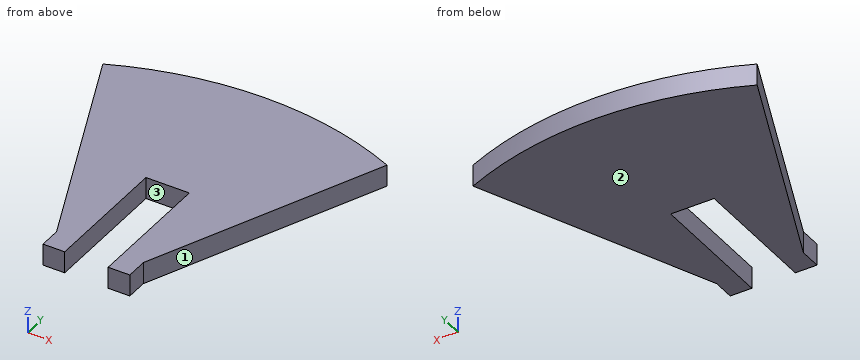
from build123d import *

# Parameters (mm, degrees)
BOSS_EXTRUDE1_DEPTH = 5
SKETCH2_W           = 20
SKETCH2_H           = 120
CUT_EXTRUDE1_DEPTH  = 10


with BuildPart() as part:
    # Sketch1 → Boss-Extrude1 (new, symmetric)
    with BuildSketch(Plane.XY):
        with BuildLine():
            Line((-65.458114903, 147.092607541), (-20, 40))
            Line((-20, 40), (-20, 30))
            Line((-20, 30), (20, 30))
            Line((20, 30), (20, 40))
            Line((20, 40), (65.458114903, 147.092607541))
            ThreePointArc((65.458114903, 147.092607541), (0, 161), (-65.458114903, 147.092607541))
        make_face()
    extrude(amount=BOSS_EXTRUDE1_DEPTH, both=True)

    # Sketch2 → Cut-Extrude1 (cut)
    with BuildSketch(Plane.XY.offset(5)):
        with Locations((0, 30)):
            Rectangle(SKETCH2_W, SKETCH2_H)
    extrude(amount=-CUT_EXTRUDE1_DEPTH, mode=Mode.SUBTRACT)


solid = part.part
Can you work these out from the model? Positions are in its coordinate system, mm. Face numbers are marked on the shaded views. Coordinates: 2 decimals unless noted, no trailing zeros. Order: outer loops, then holes, each group sorted by start corner. A loop starts at its lowest first (then second) coordinate and runs counter-clockwise, first axis right, second up. Notation, with made-up numbers: M -26,-26 L -17,-26 A20 ccw -17,-6 Z; hole C 72,-6.5 d7. An arc over 180 degrees is marked long. Write item = value, one per line.
(1) Suppose I cut it at D-D on x = -22. Please give me the cut outline in (y, z), plus the area to 3 significant figures.
Results are:
outline = M 44.71,-5 L 159.49,-5 L 159.49,5 L 44.71,5 Z
area = 1,150 mm2
(2) Suppose I cut it at A-A on y = 53. Please give me the cut outline in (x, z).
Results are:
outline = M -25.52,-5 L -10,-5 L -10,5 L -25.52,5 Z; M 10,-5 L 25.52,-5 L 25.52,5 L 10,5 Z
(3) For pin 1 Ø3 at (y, z) = (37, 1) entering from -X; pin 2 Ø3 at (y, z) = (68.5, 0.5) entering from +X; pin 3 Ø5 at (x, z) = (3, -2) entering from -Y, each with a flat end and sliding along its axis, tell me the tip position at first contact or that it passes through.
Results are:
pin_1 = -20
pin_2 = 32.73
pin_3 = 90
(4) If we mould it in two halves opening along X, with no side actions, what happens to the marked faces 1, 2 and 3? For each: pulls with the +X half, pulls with the -X half, needs draft (parallel to the pull), parting line crosses it, or undercut.
Results are:
face_1 = pulls with the +X half
face_2 = needs draft
face_3 = undercut
(5) I need wall thicknesses on line 1 along X through (y, z) = (58.5, 3.5); line 2 along X through (y, z) = (56, -0.5); line 3 along Y through (x, z) = (-14.5, -2.5). Which ranges of each line are inside material? Lowest first, please. Write a range as [from, to].
Results are:
line_1 = [-27.85, -10], [10, 27.85]
line_2 = [-26.79, -10], [10, 26.79]
line_3 = [30, 160.35]
(6) Suppose I cut it at B-B on z = 2.5. Please give me the cut outline in (x, y).
Results are:
outline = M -65.46,147.09 L -20,40 L -20,30 L -10,30 L -10,90 L 10,90 L 10,30 L 20,30 L 20,40 L 65.46,147.09 A161 ccw Z
(7) Suppose I cut it at C-C on y = 69. Please give me the cut outline in (x, z), plus the area to 3 significant figures.
Results are:
outline = M -32.31,-5 L -10,-5 L -10,5 L -32.31,5 Z; M 10,-5 L 32.31,-5 L 32.31,5 L 10,5 Z
area = 446 mm2
